```python
from build123d import *
from build123d.topology import SkipClean

# Parameters (mm, degrees)
SKETCH1_R                                            = 11
SKETCH1_R_2                                          = 8
BOSS_EXTRUDE1_DEPTH                                  = 30
BOSS_EXTRUDE2_START                                  = -14
SKETCH2_R                                            = 8
BOSS_EXTRUDE2_DEPTH                                  = 14
HOLE_SIZE_PER_SOCKET_HEAD_CAP_SCREW_TYPE_D           = 6.6
HOLE_SIZE_PER_SOCKET_HEAD_CAP_SCREW_TYPE_CBORE_D     = 15
HOLE_SIZE_PER_SOCKET_HEAD_CAP_SCREW_TYPE_CBORE_DEPTH = 9
SKETCH5_OUTSIDE_W                                    = 69.114
SKETCH5_OUTSIDE_H                                    = 37.114
SKETCH5_OUTSIDE_R                                    = 11
CUT_EXTRUDE2_DEPTH                                   = 9
CUT_EXTRUDE3_START                                   = -3
SKETCH6_R                                            = 11
CUT_EXTRUDE3_DEPTH                                   = 3
CHAMFER1_SIZE                                        = 0.5


with BuildPart() as part:
    # Sketch1 → Boss-Extrude1 (new body)
    with BuildSketch(Plane.XY):
        Circle(SKETCH1_R)
        Circle(SKETCH1_R_2, mode=Mode.SUBTRACT)
    extrude(amount=BOSS_EXTRUDE1_DEPTH)

    # Sketch2 → Boss-Extrude2 (add)
    with SkipClean():  # the faces are left unmerged after this step: merging them gives an invalid solid
        with BuildSketch(Plane.XY.offset(30).offset(BOSS_EXTRUDE2_START)):
            with BuildLine():
                Line((-21.4, 6.858571), (-2.2, 10.777755))
                ThreePointArc((-2.2, 10.777755), (0, 11), (2.2, 10.777755))
                Line((2.2, 10.777755), (21.4, 6.858571))
                ThreePointArc((21.4, 6.858571), (27, 0), (21.4, -6.858571))
                Line((21.4, -6.858571), (2.2, -10.777755))
                ThreePointArc((2.2, -10.777755), (0, -11), (-2.2, -10.777755))
                Line((-2.2, -10.777755), (-21.4, -6.858571))
                ThreePointArc((-21.4, -6.858571), (-27, 0), (-21.4, 6.858571))
            make_face()
            Circle(SKETCH2_R, mode=Mode.SUBTRACT)
        extrude(amount=BOSS_EXTRUDE2_DEPTH)

    # Hole size per socket head cap screw type1 (through all)
    with Locations(Plane(origin=(-20, 0, 30), x_dir=(1, 0, 0), z_dir=(0, 0, 1))):
        with Locations((0, 0), (40, 0)):
            CounterBoreHole(HOLE_SIZE_PER_SOCKET_HEAD_CAP_SCREW_TYPE_D / 2, HOLE_SIZE_PER_SOCKET_HEAD_CAP_SCREW_TYPE_CBORE_D / 2, HOLE_SIZE_PER_SOCKET_HEAD_CAP_SCREW_TYPE_CBORE_DEPTH)

    # Sketch5 outside → Cut-Extrude2 (cut)
    with SkipClean():  # the faces are left unmerged after this step: merging them gives an invalid solid
        with BuildSketch(Plane.XY.offset(30)):
            Rectangle(SKETCH5_OUTSIDE_W, SKETCH5_OUTSIDE_H)
            Circle(SKETCH5_OUTSIDE_R, mode=Mode.SUBTRACT)
        extrude(amount=-CUT_EXTRUDE2_DEPTH, mode=Mode.SUBTRACT)

    # Sketch6 → Cut-Extrude3 (cut)
    with SkipClean():  # the faces are left unmerged after this step: merging them gives an invalid solid
        with BuildSketch(Plane.XY.offset(30).offset(CUT_EXTRUDE3_START)):
            Circle(SKETCH6_R)
        extrude(amount=CUT_EXTRUDE3_DEPTH, mode=Mode.SUBTRACT)

    # Chamfer1
    chamfer1_edges = [part.edges().sort_by_distance(p)[0] for p in [
        (8.520563, 6.957011, 27),
        (-8, 0, 27),
        (-11, 0, 0),
        (23.3, 0, 16),
        (23.3, 0, 21),
        (-8, 0, 0),
        (-16.7, 0, 16),
        (-16.7, 0, 21),
    ]]
    chamfer(chamfer1_edges, length=CHAMFER1_SIZE)


solid = part.part
```
Verification items for the finished model (mm, model axes). Round coordinates to 2 decimals unless told otherwise and drop trailing zeros. Write each loop counter-clockwise with the first axis right and the second up, starting at its lowest first coordinate (ties: lowest second). Pieces come first, ordered by that corner, then holes. Notation, with made-up numbers: (67, -16.75) -> (113, -16.75) arc R27 cw to (113, 12.25) -> close; hole circle Ø4 at (29.25, -23). An arc over 180 degrees is marked (long way). Write each question's results on one line, items separated by ' | '. Start each with the question number.
1. Material ranges on probe 1 along Y at (x, z) = (0, 16); probe 2 along X at (y, z) = (-0.5, 19.5), recorded low to high. Write a range as from..to.
2. Cross-section at C-C (y = 0). Count the separate pieces of the cut face and the enclosed holes in it, then the cut area to 3 significant figures.
3. Draft check along Y on faces 1 (the flat face through (-11.93, 8.79, 18.46)), 2 (the cylindrical face through (-27, 0, 18)), 3 (the cylindrical face through (-23.05, -1.26, 18.47)). Enter one of: +Y half, -Y half, draft (parallel to the pull), parting line (faces both ways), or undercut.
4. Cross-section at D-D (x = 20). Enter the section's corners in (y, z), then the cut area to 3 significant figures.
5. Cross-section at B-B (z = 9.5). Enter the section's corners in (x, y), then the cut area to 3 significant figures.
6. Cross-section at A-A (x = 0). Enter the section's corners in (y, z), then the cut area to 3 significant figures.
7. Depth check by flat-ended pin: P1, Ø3, axis at y = 3.5, z = 4.5, coming from the +X side; P2, Ø10, axis at x = 12, z = 8, coming from the -Y side; P3, Ø6.5, axis at x = -16, y = 2, coming from the -Z side; P4, Ø8, axis at x = 4, z = 13, coming from the -Y side. Enter the tip coordinate at first touch or a pass-through.
Solutions:
1) probe 1: y = -11..-8, 8..11 | probe 2: x = -26.98..-23.26, -16.74..-7.98, 7.98..16.74, 23.26..26.98
2) separate pieces: 4 | enclosed holes: 0 | area: 254 mm2
3) face 1: +Y half | face 2: parting line | face 3: undercut
4) outline: (-7.14, 16) -> (-3.8, 16) -> (-3.3, 16.5) -> (-3.3, 20.5) -> (-3.8, 21) -> (-7.14, 21) -> close; (3.3, 16.5) -> (3.8, 16) -> (7.14, 16) -> (7.14, 21) -> (3.8, 21) -> (3.3, 20.5) -> close | area: 37.9 mm2
5) outline: circle Ø22 at (0, 0); hole circle Ø16 at (0, 0) | area: 179 mm2
6) outline: (-11, 0.5) -> (-10.5, 0) -> (-8.5, 0) -> (-8, 0.5) -> (-8, 26.5) -> (-8.5, 27) -> (-10.5, 27) -> (-11, 26.5) -> close; (8, 0.5) -> (8.5, 0) -> (10.5, 0) -> (11, 0.5) -> (11, 26.5) -> (10.5, 27) -> (8.5, 27) -> (8, 26.5) -> close | area: 161 mm2
7) P1: stops at x = 10.82 | P2: stops at y = -8.49 | P3: stops at z = 16 | P4: stops at y = -11
